Geometry: see drawing. Coordinates: mm, zero at the bounding-box minimum. A direction names the side the tool comes from. Give positions to 0.01 mm unless a question says otherwise; leave off trailing zeros. Write each loop counter-clockwise with the first axis right and the second up, starting at its lowest first coordinate (ties: lowest second). Pieces come first, ordered by that corner, then holes. Notation, with made-up numbers: (56.5, 27.5) - (90.5, 27.5) arc R36 ccw to (90.5, 66.5) - close; hole circle Ø4 at (-30.75, -10.5). An arc over 180 degrees is marked (long way). Use CSV: the item, a comma, the result in double quotes. Start each with the question number.
(1) Reachability of the marked faces 1, 2 and 3 from +Z, -Z, +X, -X, +Y, -Y: full face, straight path, thin tool, end or side. Return the list, or none.
(2) Section B-B on y = 16.5. Output: boundary loops of the cut face in (x, z).
(3) Section A-A on x = 25. Output: boundary loops of the cut face in (y, z), and give its area (3 significant figures).
(4) Section D-D on x = 7.5. Output: boundary loops of the cut face in (y, z).
(5) First-contact query: pin 1 Ø8 at (x, z) = (25, 105) entering from +Y; pin 2 Ø8 at (x, z) = (27.5, 99) entering from -Y; pin 3 Ø1.5 at (x, z) = (27, 31) entering from -Y. Flat tips, straight axial feed; report the tip coordinate or a pass-through.
(6) Line query: probe 1 along X at (y, z) = (19.5, 105); probe 2 along Z at (x, y) = (41, 26.5); probe 3 along X at (y, z) = (17, 58.5). Output: solid intervals per line, ascending. Write a range as [from, to].
(7) Section C-C on z = 81. Output: boundary loops of the cut face in (x, y), and give its area (3 significant figures).
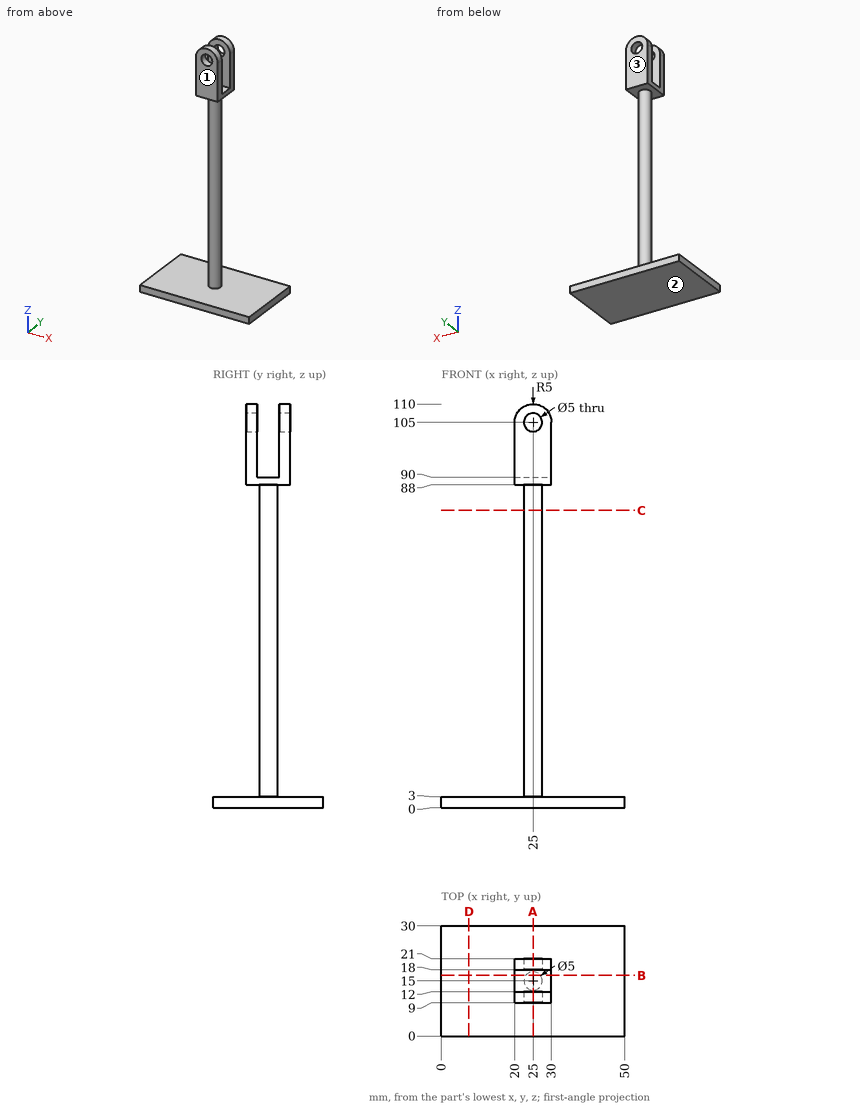
Check values:
1,face 1,"+Z, +X, -X, -Y"
1,face 2,"-Z, +X, -X, +Y, -Y"
1,face 3,"+Z, +X, -X, +Y"
2,outline,"(0, 0) - (50, 0) - (50, 3) - (27, 3) - (27, 88) - (30, 88) - (30, 90) - (20, 90) - (20, 88) - (23, 88) - (23, 3) - (0, 3) - close"
3,outline,"(0, 0) - (30, 0) - (30, 3) - (17.5, 3) - (17.5, 88) - (21, 88) - (21, 102.5) - (18, 102.5) - (18, 90) - (12, 90) - (12, 102.5) - (9, 102.5) - (9, 88) - (12.5, 88) - (12.5, 3) - (0, 3) - close; (9, 107.5) - (12, 107.5) - (12, 110) - (9, 110) - close; (18, 107.5) - (21, 107.5) - (21, 110) - (18, 110) - close"
3,area,"629 mm²"
4,outline,"(0, 0) - (30, 0) - (30, 3) - (0, 3) - close"
5,pin 1,"stops at y = 21"
5,pin 2,"stops at y = 9"
5,pin 3,"stops at y = 12.83"
6,probe 1,"x = [20, 22.5], [27.5, 30]"
6,probe 2,"z = [0, 3]"
6,probe 3,"x = [23.5, 26.5]"
7,outline,"circle Ø5 at (25, 15)"
7,area,"19.6 mm²"
